The listing builds one solid part. Answer for the finished solid, in the listing's coordinates (mm). A direction names the side the tool comes from. Give positions to 0.01 mm unless a question says otherwise; leave off trailing zeros. Order: outer loops, then holes, each group sorted by start corner. A loop starts at its lowest first (then second) coordinate and runs counter-clockwise, first axis right, second up. Notation, with made-up numbers: (48.5, 68.5) - (62.5, 68.5) arc R25 ccw to (62.5, 100.5) - close; hole circle Ø5 at (42, -19.75). An arc over 180 degrees is marked (long way). Answer in a Markdown table with one row per item.
from build123d import *

# Parameters (mm, degrees)
SLOTTED_BASE_BLOCK_DEPTH = 80
PIVOT_PAD_SKETCH_R       = 25
PIVOT_PAD_50_DEPTH       = 21
UPPER_BAR_SKETCH_W       = 30
UPPER_BAR_SKETCH_H       = 12
UPPER_BAR_DEPTH          = 100
THROUGH_SLOT_PROFILE_W   = 15
THROUGH_SLOT_PROFILE_H   = 21
THROUGH_SLOT_CUT_DEPTH   = 100
EYE_LUG_PROFILE_R        = 10
RAISED_EYE_LUG_DEPTH     = 15
LUG_SUPPORT_RIB_REACH    = 132.131
LUG_RIB_SKETCH_WALL_W    = 299.76392147
LUG_RIB_SKETCH_WALL_H    = 10
PAD_HOLE_SKETCH_R        = 10
PAD_HOLE_20_DEPTH        = 30


with BuildPart() as part:
    # Base Block Profile → Slotted Base Block (new body)
    with BuildSketch(Plane(origin=(0, 0, 0), x_dir=(0, 0, -1), z_dir=(1, 0, 0))):
        Polygon((30, 0), (-30, 0), (-30, -17), (-15, -17), (-25, -2), (25, -2), (15, -17), (30, -17), align=None)
    extrude(amount=-SLOTTED_BASE_BLOCK_DEPTH)

    # Pivot Pad Sketch → Pivot Pad Ø50 (add)
    with BuildSketch(Plane(origin=(0, 0, 0), x_dir=(1, 0, 0), z_dir=(0, 1, 0))):
        with Locations((-25, 0)):
            Circle(PIVOT_PAD_SKETCH_R)
    extrude(amount=PIVOT_PAD_50_DEPTH)

    # Upper Bar Sketch → Upper Bar (add)
    with BuildSketch(Plane(origin=(0, 0, 0), x_dir=(0, 0, -1), z_dir=(1, 0, 0))):
        with Locations((0, 6)):
            Rectangle(UPPER_BAR_SKETCH_W, UPPER_BAR_SKETCH_H)
    extrude(amount=-UPPER_BAR_DEPTH)

    # Through Slot Profile → Through Slot Cut (cut)
    with BuildSketch(Plane(origin=(0, 0, 0), x_dir=(0, 0, -1), z_dir=(1, 0, 0))):
        with Locations((-22.5, 10.5)):
            Rectangle(THROUGH_SLOT_PROFILE_W, THROUGH_SLOT_PROFILE_H)
        with Locations((22.5, 10.5)):
            Rectangle(THROUGH_SLOT_PROFILE_W, THROUGH_SLOT_PROFILE_H)
    extrude(amount=-THROUGH_SLOT_CUT_DEPTH, mode=Mode.SUBTRACT)

    # Eye Lug Profile → Raised Eye Lug (add, symmetric)
    with BuildSketch(Plane.XY):
        with BuildLine():
            Line((-85, 16), (-85, 38))
            ThreePointArc((-85, 38), (-110.606601718, 48.606601718), (-100, 23))
            Line((-100, 23), (-100, 12))
            Line((-100, 12), (-45, 12))
            Line((-45, 12), (-45, 16))
            Line((-45, 16), (-85, 16))
        make_face()
        with Locations((-100, 38)):
            Circle(EYE_LUG_PROFILE_R, mode=Mode.SUBTRACT)
    extrude(amount=RAISED_EYE_LUG_DEPTH, both=True)

    # Lug Rib Sketch wall → Lug Support Rib (add, up to next)
    with BuildSketch(Plane(origin=(-76.186743425, 31.048801232, 0), x_dir=(0.596586314149, -0.802548920484, 0), z_dir=(0.802548920484, 0.596586314149, 0)), mode=Mode.PRIVATE) as lug_support_rib_sk1:
        Rectangle(LUG_RIB_SKETCH_WALL_W, LUG_RIB_SKETCH_WALL_H)
    lug_support_rib_tool1 = extrude(lug_support_rib_sk1.sketch, amount=-LUG_SUPPORT_RIB_REACH, mode=Mode.PRIVATE) - part.part
    add(lug_support_rib_tool1.solids().sort_by_distance((-76.186743425, 31.048801232, 0))[0])

    # Pad Hole Sketch → Pad Hole Ø20 (cut)
    with BuildSketch(Plane(origin=(0, 21, 0), x_dir=(1, 0, 0), z_dir=(0, 1, 0))):
        with Locations(Location((-25, 0, 0), (0, 0, 270))):
            Circle(PAD_HOLE_SKETCH_R)
    extrude(amount=-PAD_HOLE_20_DEPTH, mode=Mode.SUBTRACT)


solid = part.part
Item 1: Each of these flat-tipped pins is pushed along its axis until it touches: P1, Ø16.5, axis at x = -55, z = -23, coming from the +Y side; P2, Ø5.5, axis at x = -1.5, z = 7, coming from the +Y side; P3, Ø18, axis at x = -25, z = 0, coming from the -Y side; P4, Ø3, axis at y = 32, z = -9, coming from the +X side. Where does it stop, or does it pass through?
Answer block:
| item | result |
|---|---|
| P1 | y = 16 |
| P2 | y = 21 |
| P3 | through |
| P4 | x = -85 |
Item 2: Consider line 1 (X direction, y = 3, z = 0); line 2 (X direction, y = 17, z = 6.5); line 3 (Y direction, x = -36.5, z = -4). Determine where each line is inside the solid, lowest interval first.
Answer block:
| item | result |
|---|---|
| line 1 | -100 to -35, -15 to 0 |
| line 2 | -100 to -85, -49.14 to -32.6, -17.4 to -0.86 |
| line 3 | -2 to 21 |
Item 3: Determine the mould class of faces 1 (the face through (0, 1, 0)), 2 (the face through (-77, 25, 5)), 3 (the face through (-90, 0, 0)) for opening direction X: pulls with the +X half, pulls with the -X half, needs draft (parallel to the pull), parting line crosses it, or undercut.
Answer block:
| item | result |
|---|---|
| face 1 | pulls with the +X half |
| face 2 | undercut |
| face 3 | needs draft |
Item 4: Find section D-D on y = -4. Write down the section's boundary in (x, z).
Answer block:
| item | result |
|---|---|
| outline | (-80, -30) - (0, -30) - (0, -23.67) - (-80, -23.67) - close; (-80, 23.67) - (0, 23.67) - (0, 30) - (-80, 30) - close |
Item 5: Find section A-A on z = 20.5. Write down the section's boundary in (x, y), then the cut area to 3 significant figures.
Answer block:
| item | result |
|---|---|
| outline | (-80, -17) - (0, -17) - (0, -8.75) - (-80, -8.75) - close; (-80, -2) - (0, -2) - (0, 0) - (-80, 0) - close |
| area | 820 mm² |
Item 6: Find section B-B on z = 6.5. Write down the section's boundary in (x, y), then the cut area to 3 significant figures.
Answer block:
| item | result |
|---|---|
| outline | (-100, 0) - (-80, 0) - (-80, -2) - (-32.6, -2) - (-32.6, 21) - (-49.14, 21) - (-49.14, 16) - (-85, 16) - (-85, 38) arc R15 ccw (long way) to (-100, 23) - close; (-17.4, -2) - (0, -2) - (0, 12) - (-0.86, 12) - (-0.86, 21) - (-17.4, 21) - close; hole circle Ø20 at (-100, 38) |
| area | 2,190 mm² |
Item 7: Which of the six approach directions +Z, -Z, +X, -X, +Y, -Y give full straight-line access (tool end or side, diameter ignored) to faces 4 (the face through (-39, -2, 0)), 5 (the face through (-100, 12, 0)), 6 (the face through (-39, 0, -23)), 7 (the face through (-77, 25, -5))?
Answer block:
| item | result |
|---|---|
| face 4 | +X, -X |
| face 5 | +Z, -Z, -X, -Y |
| face 6 | -Z, +X, -X, +Y |
| face 7 | -Z, +Y |
Item 8: Find section C-C on x = -25. Write down the section's boundary in (y, z), then the cut area to 3 significant figures.
Answer block:
| item | result |
|---|---|
| outline | (-17, -30) - (0, -30) - (0, -15) - (21, -15) - (21, -10) - (-2, -10) - (-2, -25) - (-17, -15) - close; (-17, 15) - (-2, 25) - (-2, 10) - (21, 10) - (21, 15) - (0, 15) - (0, 30) - (-17, 30) - close |
| area | 590 mm² |
